```python
from build123d import *

# Parameters (mm, degrees)
SKETCH1_W           = 320
SKETCH1_H           = 30
BOSS_EXTRUDE1_DEPTH = 10
CHAMFER1_SIZE       = 2
M6_TAPPED_HOLE1_D   = 5
HOLE1_D             = 6.6
HOLE1_CBORE_D       = 11
HOLE1_CBORE_DEPTH   = 6.8


with BuildPart() as part:
    # Sketch1 → Boss-Extrude1 (new body)
    with BuildSketch(Plane.XY):
        Rectangle(SKETCH1_W, SKETCH1_H)
    extrude(amount=BOSS_EXTRUDE1_DEPTH)

    # Chamfer1
    chamfer1_edges = [part.edges().sort_by_distance(p)[0] for p in [
        (160, -15, 5),
        (-160, -15, 5),
        (-160, 15, 5),
        (160, 15, 5),
    ]]
    chamfer(chamfer1_edges, length=CHAMFER1_SIZE)

    # M6 Tapped Hole1 (through all)
    with Locations(Plane.XY.offset(10)):
        with Locations((-139.5, -9), (-46.5, -9), (46.5, -9), (139.5, -9)):
            Hole(M6_TAPPED_HOLE1_D / 2)

    # Hole1 (through all)
    with Locations(Plane.XY.offset(10)):
        with Locations((-95, 5), (95, 5)):
            CounterBoreHole(HOLE1_D / 2, HOLE1_CBORE_D / 2, HOLE1_CBORE_DEPTH)


solid = part.part
```
Geometry: final body of the model. Coordinates: model frame, mm. A direction names the side the tool comes from. Coordinates: 2 decimals unless noted, no trailing zeros. Loops run counter-clockwise (first coordinate to the right, second up) from the corner with the lowest first, then second, coordinate; pieces in that order, holes last. Notation, with made-up numbers: (-21.5, 72) -> (-6.5, 72) arc R9 ccw to (-6.5, 86) -> close; hole circle Ø1 at (-9, 47.25). An arc over 180 degrees is marked (long way). Use a Markdown table: item, result. Add a question column.
(1) Section query C-C, the plane z = 5.75. Return loops of the section in (x, y), plus the area to 3 significant figures.
(2) Section query B-B, the plane x = 95. Return loops of the section in (y, z).
(3) Access query for faces 4 (the cylindrical face through (-100.495, 5.242, 6.648)), 5 (the cylindrical face through (44.19, -9.96, 4.93)). Directions: +Z, -Z, +X, -X, +Y, -Y. A direction counts if a zero-diameter tool reaches every point of the face in a straight line with its end or side. Return the directions, or none.
(4) Section query A-A, the plane y = 5. Return loops of the section in (x, z), plus the area to 3 significant figures.
(5) Line query: line 1 along X through (y, z) = (-9.25, 3.5); line 2 along Y through (x, z) = (-95, 5.25); line 3 along Y through (x, z) = (-46.5, 3). Output: solid intervals per line, ascending.
(6) Pin query (flat end, axial travel): pin 1 Ø3.5 at (x, y) = (-95, 3.5) entering from +Z; pin 2 Ø5.5 at (x, y) = (95.5, 3) entering from +Z. Return the tip coordinate at first contact, or that it passes through.
(7) Mould query, pull axis Y, two halves, no side actions, for faces 1 (the cylindrical face through (89.505, 5.242, 6.648)), 2 (the flat face through (-2, 0, 10)), 3 (the flat face through (-2, 15, 5)). Classes: pulls with the +Y half, pulls with the -Y half, needs draft (parallel to the pull), parting line crosses it, or undercut.
Answer:
| question | item | result |
|---|---|---|
| 1 | outline | (-160, -13) -> (-158, -15) -> (158, -15) -> (160, -13) -> (160, 13) -> (158, 15) -> (-158, 15) -> (-160, 13) -> close; hole circle Ø5 at (-139.5, -9); hole circle Ø11 at (-95, 5); hole circle Ø5 at (-46.5, -9); hole circle Ø5 at (46.5, -9); hole circle Ø11 at (95, 5); hole circle Ø5 at (139.5, -9) |
| 1 | area | 9,320 mm^2 |
| 2 | outline | (-15, 0) -> (1.7, 0) -> (1.7, 3.2) -> (-0.5, 3.2) -> (-0.5, 10) -> (-15, 10) -> close; (8.3, 0) -> (15, 0) -> (15, 10) -> (10.5, 10) -> (10.5, 3.2) -> (8.3, 3.2) -> close |
| 3 | face 4 | +Z |
| 3 | face 5 | +Z, -Z |
| 4 | outline | (-160, 0) -> (-98.3, 0) -> (-98.3, 3.2) -> (-100.5, 3.2) -> (-100.5, 10) -> (-160, 10) -> close; (-91.7, 0) -> (91.7, 0) -> (91.7, 3.2) -> (89.5, 3.2) -> (89.5, 10) -> (-89.5, 10) -> (-89.5, 3.2) -> (-91.7, 3.2) -> close; (98.3, 0) -> (160, 0) -> (160, 10) -> (100.5, 10) -> (100.5, 3.2) -> (98.3, 3.2) -> close |
| 4 | area | 3,010 mm^2 |
| 5 | line 1 | x = -160 to -141.99, -137.01 to -48.99, -44.01 to 44.01, 48.99 to 137.01, 141.99 to 160 |
| 5 | line 2 | y = -15 to -0.5, 10.5 to 15 |
| 5 | line 3 | y = -15 to -11.5, -6.5 to 15 |
| 6 | pin 1 | passes through |
| 6 | pin 2 | stops at z = 3.2 |
| 7 | face 1 | undercut |
| 7 | face 2 | needs draft |
| 7 | face 3 | pulls with the +Y half |
